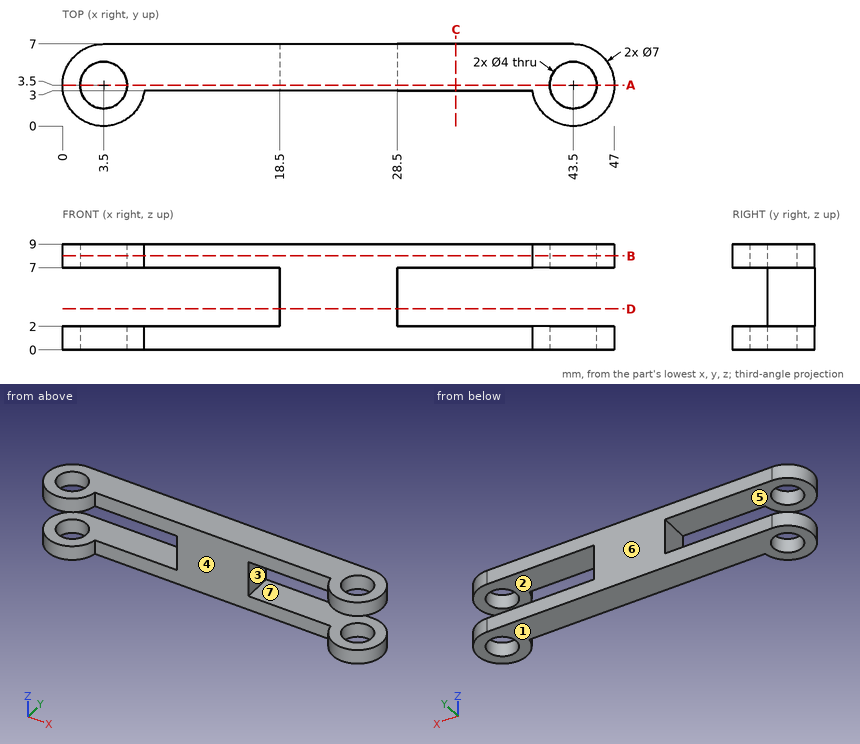
Input: dimensioned drawing with shaded views. Units: mm. Origin: part minimum x, y, z. A direction names the side the tool comes from. Give positions to 0.01 mm unless a question says otherwise; leave off trailing zeros. Loops run counter-clockwise (first coordinate to the right, second up) from the corner with the lowest first, then second, coordinate; pieces in that order, holes last. Notation, with made-up numbers: M -6,20.25 L 6,20.25 A21 cw 6,50.25 Z; hole C 71,-31 d7. An arc over 180 degrees is marked long. Put each result on its own line as item: value. Start each with the question number.
1) Cut plane B-B (z = 8). Output: boundary loops of the cut face in (x, y), then the cut area to 3 significant figures.
2) Contact query for flat-ended pins moving along their axis: pin 1 (3 mm diameter, centred on y = 6, z = 4.5, fed in from +X); pin 2 (2.5 mm diameter, centred on x = 26.5, z = 5.5, fed in from -Y). Output: stop coordinate, or through.
3) Cut plane A-A (y = 3.5). Output: boundary loops of the cut face in (x, z).
4) Access query for the marked faces 5, 6 and 7. Directions: +Z, -Z, +X, -X, +Y, -Y. A direction counts if a zero-diameter tool reaches every point of the face in a straight line with its end or side. Return the directions, or none.
5) Cut plane C-C (x = 33.5). Output: boundary loops of the cut face in (y, z).
6) Cut plane D-D (z = 3.5). Output: boundary loops of the cut face in (x, y).
7) Ray query, line 1 along X through (y, z) = (3.5, 7.6); line 2 along Z through (x, y) = (2, 0.75); line 3 along Y through (x, z) = (43.5, 8.35). Return the intervals inside material, ascending.
8) Pull-direction query (Z, two-part tool) for the marked faces 1, 2, 3 and 4; classes: pulls with the +Z half, pulls with the -Z half, needs draft (parallel to the pull), parting line crosses it, or undercut.
Verdict:
1. outline: M 3.5,7 A3.5 ccw long 6.96,3 L 40.04,3 A3.5 ccw long 43.5,7 Z; hole C 3.5,3.5 d4; hole C 43.5,3.5 d4
1. area: 189 mm2
2. pin 1: x = 28.5
2. pin 2: y = 3
3. outline: M 0,0 L 1.5,0 L 1.5,2 L 0,2 Z; M 0,7 L 1.5,7 L 1.5,9 L 0,9 Z; M 5.5,0 L 41.5,0 L 41.5,2 L 28.5,2 L 28.5,7 L 41.5,7 L 41.5,9 L 5.5,9 L 5.5,7 L 18.5,7 L 18.5,2 L 5.5,2 Z; M 45.5,0 L 47,0 L 47,2 L 45.5,2 Z; M 45.5,7 L 47,7 L 47,9 L 45.5,9 Z
4. face 5: -X, +Y, -Y
4. face 6: +Z, -Z, +X, -X, +Y
4. face 7: +X, +Y, -Y
5. outline: M 3,0 L 7,0 L 7,2 L 3,2 Z; M 3,7 L 7,7 L 7,9 L 3,9 Z
6. outline: M 18.5,3 L 28.5,3 L 28.5,7 L 18.5,7 Z
7. line 1: 0 to 1.5, 5.5 to 41.5, 45.5 to 47
7. line 2: 0 to 2, 7 to 9
7. line 3: 0 to 1.5, 5.5 to 7
8. face 1: pulls with the -Z half
8. face 2: undercut
8. face 3: undercut
8. face 4: needs draft
